Here's the drawing with two shaded views (mm, measured from the low corner). I have some questions. Coordinates: 2 decimals unless noted, no trailing zeros. Write each loop counter-clockwise with the first axis right and the second up, starting at its lowest first coordinate (ties: lowest second). Pieces come first, ordered by that corner, then holes.
Item 1: If we section it at B-B (x = 46): Please give me the cut outline in (y, z), then the cut area to 3 significant figures.
Item 2: If we section it at A-A (z = 90): Please give me the cut outline in (x, y).
Item 3: If we section it at D-D (z = 42.5): Please give me the cut outline in (x, y).
Item 4: I'm going to push a flat-ended pin straight in: pin 1 Ø3 at (x, z) = (52.57, 31.43) entering from -Y. Where does the tip first touch, or does it pass through?
Item 5: If we section it at C-C (y = 4.5): Count the separate pieces of the cut face and the enclosed holes in it, then the cut area to 3 significant figures.
Item 6: If I drill on line 1 (X direction, y = 4.25, z = 90); line 2 (X direction, y = 3.75, z = 8.5) (3 decimals); line 3 (Z direction, x = 38, y = 1.75), over which ranges is the centre line in solid material (lowest first)?
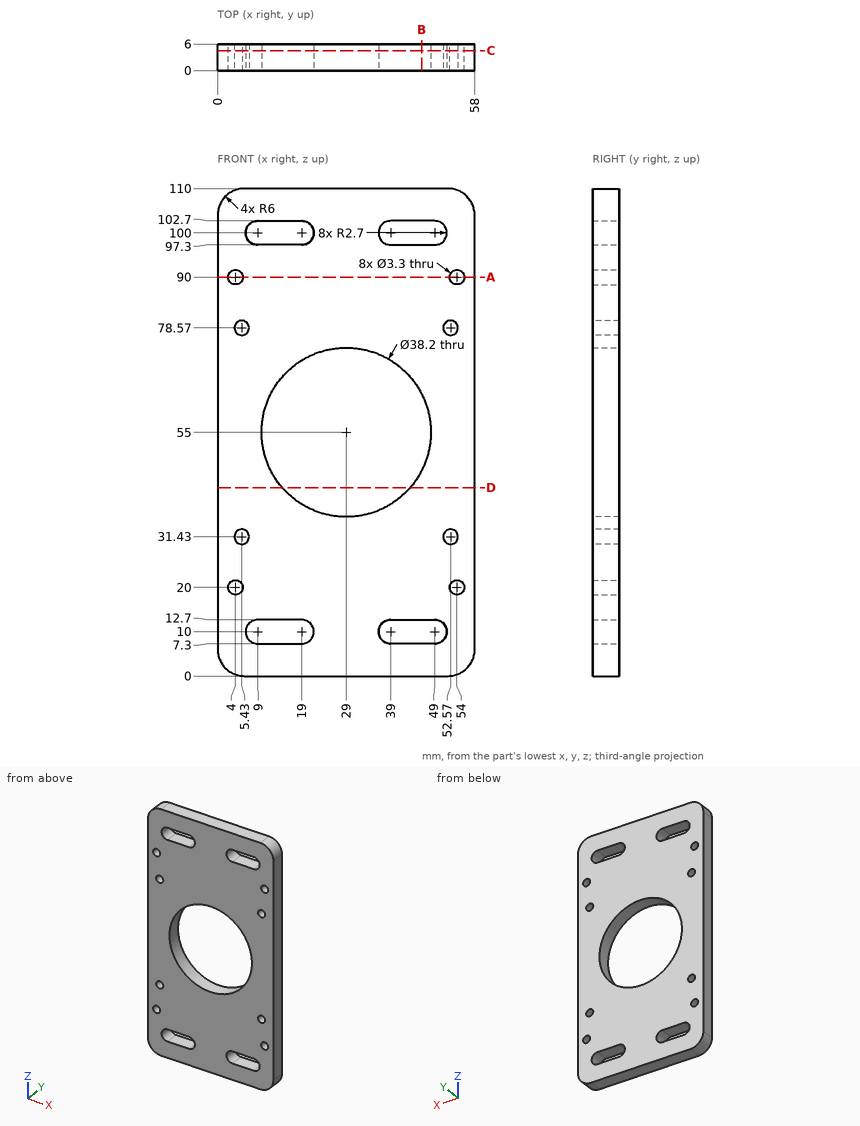
Answer list:
1. outline: (0, 0) - (6, 0) - (6, 7.3) - (0, 7.3) - close; (0, 12.7) - (6, 12.7) - (6, 46.29) - (0, 46.29) - close; (0, 63.71) - (6, 63.71) - (6, 97.3) - (0, 97.3) - close; (0, 102.7) - (6, 102.7) - (6, 110) - (0, 110) - close
1. area: 491 mm2
2. outline: (0, 0) - (2.35, 0) - (2.35, 6) - (0, 6) - close; (5.65, 0) - (52.35, 0) - (52.35, 6) - (5.65, 6) - close; (55.65, 0) - (58, 0) - (58, 6) - (55.65, 6) - close
3. outline: (0, 0) - (14.56, 0) - (14.56, 6) - (0, 6) - close; (43.44, 0) - (58, 0) - (58, 6) - (43.44, 6) - close
4. pin 1: passes through
5. separate pieces: 1
5. enclosed holes: 13
5. area: 4,830 mm2
6. line 1: x = 0 to 2.35, 5.65 to 52.35, 55.65 to 58
6. line 2: x = 0 to 6.755, 21.245 to 36.755, 51.245 to 58
6. line 3: z = 0 to 7.49, 12.51 to 38.15, 71.85 to 97.49, 102.51 to 110
